from build123d import *

# Parameters (mm, degrees)
BOSS_EXTRUDE1_DEPTH = 10
SKETCH2_R           = 10
CUT_EXTRUDE1_DEPTH  = 157.604597634
SKETCH3_R           = 10
CUT_EXTRUDE2_DEPTH  = 10


with BuildPart() as part:
    # Sketch1 → Boss-Extrude1 (new body)
    with BuildSketch(Plane.XY):
        with BuildLine():
            Line((-135, 20), (135, 20))
            ThreePointArc((135, 20), (155, 0), (135, -20))
            Line((135, -20), (-135, -20))
            ThreePointArc((-135, -20), (-155, 0), (-135, 20))
        make_face()
    extrude(amount=BOSS_EXTRUDE1_DEPTH)

    # Sketch2 → Cut-Extrude1 (cut, through all)
    with BuildSketch(Plane.XY.offset(10)):
        with Locations((-135, 0)):
            Circle(SKETCH2_R)
        with Locations((135, 0)):
            Circle(SKETCH2_R)
    extrude(amount=-CUT_EXTRUDE1_DEPTH, mode=Mode.SUBTRACT)

    # Sketch3 → Cut-Extrude2 (cut)
    with BuildSketch(Plane.XY.offset(10)):
        Circle(SKETCH3_R)
    extrude(amount=-CUT_EXTRUDE2_DEPTH, mode=Mode.SUBTRACT)


solid = part.part
Model file for the job. Use its own axes, mm. Give positions to 0.01 mm unless a question says otherwise; leave off trailing zeros. Order: outer loops, then holes, each group sorted by start corner. A loop starts at its lowest first (then second) coordinate and runs counter-clockwise, first axis right, second up. Notation, with made-up numbers: (-17.5, 13.5) - (16.5, 13.5) arc R21 ccw to (16.5, 38.5) - close; hole circle Ø10 at (86, 4.5). An arc over 180 degrees is marked (long way). Return JSON: item names as keys, results as strings.
1) Cut at A-A, the plane y = 0. Give the cut face in (x, z).
Geometry says:
{"outline": "(-155, 0) - (-145, 0) - (-145, 10) - (-155, 10) - close; (-125, 0) - (-10, 0) - (-10, 10) - (-125, 10) - close; (10, 0) - (125, 0) - (125, 10) - (10, 10) - close; (145, 0) - (155, 0) - (155, 10) - (145, 10) - close"}
2) Probe line 1 (Y direction, x = 135, z = 4.5); line 2 (X direction, y = 8, z = 5.5); line 3 (X direction, y = 2, z = 3.25). List the from-to ranges inside material, lowest first. Write a range as from..to.
Geometry says:
{"line 1": "-20..-10, 10..20", "line 2": "-153.33..-141, -129..-6, 6..129, 141..153.33", "line 3": "-154.9..-144.8, -125.2..-9.8, 9.8..125.2, 144.8..154.9"}
3) Cut at C-C, the plane y = 13. Give the cut face in (x, z), plus the area to 3 significant figures.
Geometry says:
{"outline": "(-150.2, 0) - (150.2, 0) - (150.2, 10) - (-150.2, 10) - close", "area": "3,000 mm²"}
4) Pull direction X, two halves, no side cores. Call faces 1 (the cylindrical face through (-125.763, -3.83, 5.07)), 2 (the cylindrical face through (155, 0, 5)), 3 (the flat face through (2, 14, 10)): pulls with the +X half, pulls with the -X half, needs draft (parallel to the pull), parting line crosses it, or undercut.
Geometry says:
{"face 1": "undercut", "face 2": "pulls with the +X half", "face 3": "needs draft"}
5) Cut at B-B, the plane z = 8.5. Give the cut face in (x, y).
Geometry says:
{"outline": "(-135, -20) - (135, -20) arc R20 ccw to (135, 20) - (-135, 20) arc R20 ccw to start; hole circle Ø20 at (-135, 0); hole circle Ø20 at (0, 0); hole circle Ø20 at (135, 0)"}
6) Flat gauge pins, fed straight in: P1, Ø1, axis at y = 12, z = 1, coming from the -X side; P2, Ø3, axis at y = 7, z = 6.5, coming from the +X side; P3, Ø5, axis at y = -14, z = 7.5, coming from the +X side. Where does each tip first touch, or does it go through?
Geometry says:
{"P1": "x = -151.36", "P2": "x = 154.23", "P3": "x = 151.36"}
